The model under review builds one solid part; all positions refer to its coordinate system, in mm. A direction names the side the tool comes from. Give positions to 0.01 mm unless a question says otherwise; leave off trailing zeros. Order: outer loops, then holes, each group sorted by start corner. A loop starts at its lowest first (then second) coordinate and runs counter-clockwise, first axis right, second up. Notation, with made-up numbers: M -25.75,-26.5 L 7.25,-26.5 A21 cw 7.25,1.5 Z; hole C 52.5,-26 d10. An arc over 180 degrees is marked long. One line per question, with ' | ' between items. Start each with the question number.
1. We need section B-B on y = 15. Write out the cut boundary in (x, z).
2. We need section A-A on z = 12.5. Write out the cut boundary in (x, y), then the cut area to 3 significant figures.
3. Wall thickness on L1, parallel to X at y = 9, z = 12; L2, parallel to Y at x = 42.5, z = -38; L3, parallel to Y at x = -42, z = -26: over which ranges is each line inside the solid? List them lowest first.
4. We need section D-D on y = 107. Write out the cut boundary in (x, z).
5. For faces 5 (the face through (38.92, 145.266, -36.248)), 6 (the face through (-59, 65, -18.5)), 7 (the face through (15, 111, -37)), list the 3-axis set-ups (+Z, -Z, +X, -X, +Y, -Y) from which the entire face can be reached by the end or side of a thin tool; tool diameter is ignored.
6. The part is to be moulded in two halves that separate along X. For faces 1 (the face through (1, 3, 0)), 2 (the face through (-43.9, 65.56, -30.33)), 3 (the face through (42.932, 10.605, 11.459)), 4 (the face through (-28.901, 77.367, -36.584)), say which applies: +X half, -X half, draft (parallel to the pull), parting line (faces both ways), or undercut.
7. We need section C-C on x = -53. Write out the cut boundary in (y, z).
8. Insertion check: P1, Ø22, axis at x = 25.5, z = 9, coming from the +Y side; P2, Ø12, axis at x = 22.5, y = 20.5, coming from the -Z side; P3, Ø21, axis at x = 35, z = 12.5, coming from the -Y side. Each pin has a flat end and moves straight along its axis. Give the tip position at first contact, or say it passes through.
```python
from build123d import *

# Parameters (mm, degrees)
BASE_PLATE_SKETCH_W              = 140
BASE_PLATE_SKETCH_H              = 85
BASE_PLATE_85X140X18_DEPTH       = 18
UNDERSIDE_GROOVE_SKETCH_W        = 49
UNDERSIDE_GROOVE_SKETCH_H        = 3
UNDERSIDE_GROOVE_DEPTH           = 140
UPRIGHT_WALL_SKETCH_W            = 140
UPRIGHT_WALL_SKETCH_H            = 12
UPRIGHT_WALL_DEPTH               = 100
SMALL_LUG_40_SKETCH_R            = 20
SMALL_LUG_40_DEPTH               = 12
LARGE_LUG_55_SKETCH_R            = 27.5
LARGE_LUG_55_DEPTH               = 24
LARGE_START                      = 12
LARGE_LUG_EXTENSION_SKETCH_R     = 27.5
LARGE_LUG_EXTENSION_DEPTH        = 12
LUG_START                        = -12
LUG_RELIEF_CUT_DEPTH             = 12
LARGE_LUG_BORE_30_SKETCH_R       = 15
LARGE_LUG_BORE_30_DEPTH          = 36
SMALL_LUG_BORE_SKETCH_R          = 11.34199473
SMALL_LUG_BORE_DEPTH             = 36
BASE_MOUNTING_HOLE_1_16_SKETCH_R = 8
BASE_MOUNTING_HOLE_1_16_DEPTH    = 15
BASE_MOUNTING_HOLE_2_16_SKETCH_R = 8
BASE_MOUNTING_HOLE_2_16_DEPTH    = 15


with BuildPart() as part:
    # Base Plate Sketch → Base Plate 85x140x18 (new body)
    with BuildSketch(Plane(origin=(0, 0, 0), x_dir=(1, 0, 0), z_dir=(0, 1, 0))):
        Rectangle(BASE_PLATE_SKETCH_W, BASE_PLATE_SKETCH_H)
    extrude(amount=BASE_PLATE_85X140X18_DEPTH)

    # Underside Groove Sketch → Underside Groove (cut)
    with BuildSketch(Plane(origin=(70, 0, 0), x_dir=(0, 0, -1), z_dir=(1, 0, 0))):
        with Locations((0, 1.5)):
            Rectangle(UNDERSIDE_GROOVE_SKETCH_W, UNDERSIDE_GROOVE_SKETCH_H)
    extrude(amount=-UNDERSIDE_GROOVE_DEPTH, mode=Mode.SUBTRACT)

    # Upright Wall Sketch → Upright Wall (add)
    with BuildSketch(Plane(origin=(0, 18, 0), x_dir=(1, 0, 0), z_dir=(0, 1, 0))):
        with Locations((0, 36.5)):
            Rectangle(UPRIGHT_WALL_SKETCH_W, UPRIGHT_WALL_SKETCH_H)
    extrude(amount=UPRIGHT_WALL_DEPTH)

    # Small Lug Ø40 Sketch → Small Lug Ø40 (add)
    with BuildSketch(Plane.XY.offset(-30.5)):
        with Locations(Location((-50, 56, 0), (0, 0, 180))):
            Circle(SMALL_LUG_40_SKETCH_R)
    extrude(amount=SMALL_LUG_40_DEPTH)

    # Large Lug Ø55 Sketch → Large Lug Ø55 (add)
    with BuildSketch(Plane.XY.offset(-30.5)):
        with Locations((42.5, 118)):
            Circle(LARGE_LUG_55_SKETCH_R)
    extrude(amount=-LARGE_LUG_55_DEPTH)

    # Large Lug Extension Sketch → Large Lug Extension (add)
    with BuildSketch(Plane.XY.offset(-30.5).offset(LARGE_START)):
        with Locations((42.5, 118)):
            Circle(LARGE_LUG_EXTENSION_SKETCH_R)
    extrude(amount=-LARGE_LUG_EXTENSION_DEPTH)

    # Lug Relief Cut Sketch → Lug Relief Cut (cut)
    with BuildSketch(Plane.XY.offset(-30.5).offset(LUG_START)):
        with BuildLine():
            Line((15, 118), (15, 103.64309486))
            ThreePointArc((15, 103.64309486), (8.240000897, 86.546242306), (-8.384189381, 78.695366386))
            Line((-8.384189381, 78.695366386), (-50, 76))
            ThreePointArc((-50, 76), (-64.142135624, 70.142135624), (-70, 56))
            Line((-70, 56), (-70, 118))
            Line((-70, 118), (15, 118))
        make_face()
    extrude(amount=LUG_RELIEF_CUT_DEPTH, mode=Mode.SUBTRACT)

    # Large Lug Bore Ø30 Sketch → Large Lug Bore Ø30 (cut)
    with BuildSketch(Plane.XY.offset(-18.5)):
        with Locations((42.5, 118)):
            Circle(LARGE_LUG_BORE_30_SKETCH_R)
    extrude(amount=-LARGE_LUG_BORE_30_DEPTH, mode=Mode.SUBTRACT)

    # Small Lug Bore Sketch → Small Lug Bore (cut)
    with BuildSketch(Plane.XY.offset(-18.5)):
        with Locations((-50, 56)):
            Circle(SMALL_LUG_BORE_SKETCH_R)
    extrude(amount=-SMALL_LUG_BORE_DEPTH, mode=Mode.SUBTRACT)

    # Base Mounting Hole 1 Ø16 Sketch → Base Mounting Hole 1 Ø16 (cut)
    with BuildSketch(Plane(origin=(0, 18, 0), x_dir=(1, 0, 0), z_dir=(0, 1, 0))):
        with Locations(Location((-35, -12.5, 0), (0, 0, 270))):
            Circle(BASE_MOUNTING_HOLE_1_16_SKETCH_R)
    extrude(amount=-BASE_MOUNTING_HOLE_1_16_DEPTH, mode=Mode.SUBTRACT)

    # Base Mounting Hole 2 Ø16 Sketch → Base Mounting Hole 2 Ø16 (cut)
    with BuildSketch(Plane(origin=(0, 18, 0), x_dir=(1, 0, 0), z_dir=(0, 1, 0))):
        with Locations(Location((35, -12.5, 0), (0, 0, 270))):
            Circle(BASE_MOUNTING_HOLE_2_16_SKETCH_R)
    extrude(amount=-BASE_MOUNTING_HOLE_2_16_DEPTH, mode=Mode.SUBTRACT)


solid = part.part
```
Entries:
1) outline: M -70,-42.5 L 70,-42.5 L 70,42.5 L -70,42.5 Z; hole C -35,12.5 d16; hole C 35,12.5 d16
2) outline: M -70,3 L -43,3 L -43,18 L -70,18 Z; M -27,3 L 27,3 L 27,18 L -27,18 Z; M 43,3 L 70,3 L 70,18 L 43,18 Z | area: 1,620 mm^2
3) L1: x = -70 to -42.98, -27.02 to 27.02, 42.98 to 70 | L2: y = 0 to 103, 133 to 145.5 | L3: y = 0 to 18, 37.67 to 47.96, 64.04 to 74.33
4) outline: M 15,-42.5 L 17.3,-42.5 L 17.3,-54.5 L 32.3,-54.5 L 32.3,-18.5 L 17.3,-18.5 L 17.3,-30.5 L 15,-30.5 Z; M 52.7,-54.5 L 67.7,-54.5 L 67.7,-42.5 L 70,-42.5 L 70,-30.5 L 67.7,-30.5 L 67.7,-18.5 L 52.7,-18.5 Z
5) face 5: none | face 6: +Z, +X, -X, +Y | face 7: +Z, -Z, -X, +Y
6) face 1: draft | face 2: undercut | face 3: undercut | face 4: -X half
7) outline: M 0,-42.5 L 45.06,-42.5 L 45.06,-18.5 L 36.23,-18.5 L 36.23,-30.5 L 18,-30.5 L 18,42.5 L 0,42.5 L 0,24.5 L 3,24.5 L 3,-24.5 L 0,-24.5 Z; M 66.94,-42.5 L 75.77,-42.5 L 75.77,-18.5 L 66.94,-18.5 Z
8) P1: stops at y = 18 | P2: stops at z = -42.5 | P3: stops at y = 3
